The model under review builds one solid part; all positions refer to its coordinate system, in mm. A direction names the side the tool comes from. Coordinates: 2 decimals unless noted, no trailing zeros. Loops run counter-clockwise (first coordinate to the right, second up) from the corner with the lowest first, then second, coordinate; pieces in that order, holes last. Notation, with made-up numbers: M 61,60 L 76,60 A20 cw 76,97 Z; hole C 69,28.5 d7. An arc over 180 degrees is marked long. One line per item, written item: value.
```python
from build123d import *

# Parameters (mm, degrees)
BASE_PLATE_SKETCH_W        = 154
BASE_PLATE_SKETCH_H        = 154
BASE_PLATE_DEPTH           = 25
PLATE_CORNER_FILLETS_R26_R = 26
CORNER_HOLES_SKETCH_R      = 10
CORNER_HOLES_4X_20_DEPTH   = 25
CENTRAL_HUB_BOSS_DEPTH     = 31
CENTRE_TAP_DRILL_M20X2_0_D = 18
COUNTERBORE_SKETCH_R       = 14
COUNTERBORE_28_DEPTH       = 225.873297659
BORE_STEP_SKETCH_R         = 20
BORE_STEP_CUT_DEPTH        = 26
LUG_SLOT_A_SKETCH_R        = 5
LUG_SLOT_A_DEPTH           = 190.915770804
LUG_SLOT_B_SKETCH_R        = 5
LUG_SLOT_B_DEPTH           = 190.915770804
HUB_FILLETS_R12_R          = 12


with BuildPart() as part:
    # Base Plate Sketch → Base Plate (new body)
    with BuildSketch(Plane.XY):
        with Locations((77, 77)):
            Rectangle(BASE_PLATE_SKETCH_W, BASE_PLATE_SKETCH_H)
    extrude(amount=BASE_PLATE_DEPTH)

    # Plate Corner Fillets R26
    plate_corner_fillets_r26_edges = [part.edges().sort_by_distance(p)[0] for p in [
        (0, 154, 12.5),
        (154, 154, 12.5),
        (154, 0, 12.5),
        (0, 0, 12.5),
    ]]
    fillet(plate_corner_fillets_r26_edges, radius=PLATE_CORNER_FILLETS_R26_R)

    # Corner Holes Sketch → Corner Holes 4xØ20 (cut)
    with BuildSketch(Plane.XY.offset(25)):
        with Locations((26, 128)):
            Circle(CORNER_HOLES_SKETCH_R)
        with Locations((128, 128)):
            Circle(CORNER_HOLES_SKETCH_R)
        with Locations((128, 26)):
            Circle(CORNER_HOLES_SKETCH_R)
        with Locations((26, 26)):
            Circle(CORNER_HOLES_SKETCH_R)
    extrude(amount=-CORNER_HOLES_4X_20_DEPTH, mode=Mode.SUBTRACT)

    # Hub Profile Sketch → Central Hub Boss (add)
    with BuildSketch(Plane.XY.offset(25)):
        with BuildLine():
            Line((14, 58), (51.135796279, 58))
            Line((51.135796279, 58), (59.2634951, 27.931385667))
            Line((59.2634951, 27.931385667), (60.132879108, 24.715078934))
            ThreePointArc((60.132879108, 24.715078934), (77.84706214, 13.019941999), (94.383283675, 26.328656654))
            Line((94.383283675, 26.328656654), (102.894202658, 58))
            Line((102.894202658, 58), (140, 58))
            Line((140, 58), (140, 68))
            Line((140, 68), (108, 68))
            Line((108, 68), (108, 77))
            Line((108, 77), (108, 86))
            Line((108, 86), (140, 86))
            Line((140, 86), (140, 96))
            Line((140, 96), (102.894202658, 96))
            Line((102.894202658, 96), (94.383283675, 127.671343346))
            ThreePointArc((94.383283675, 127.671343346), (76.094284636, 140.977198883), (59.23523482, 125.900537557))
            Line((59.23523482, 125.900537557), (51.142468246, 96))
            Line((51.142468246, 96), (14, 96))
            Line((14, 96), (14, 86))
            Line((14, 86), (46, 86))
            Line((46, 86), (46, 77))
            Line((46, 77), (46, 68))
            Line((46, 68), (14, 68))
            Line((14, 68), (14, 58))
        make_face()
    extrude(amount=CENTRAL_HUB_BOSS_DEPTH)

    # Centre Tap Drill M20x2.0 (through all)
    with Locations(Plane.XY.offset(56)):
        with Locations((77, 123), (77, 31)):
            Hole(CENTRE_TAP_DRILL_M20X2_0_D / 2)

    # Counterbore Sketch → Counterbore Ø28 (cut, through all)
    with BuildSketch(Plane.XY.offset(56)):
        with Locations((77, 77)):
            Circle(COUNTERBORE_SKETCH_R)
    extrude(amount=-COUNTERBORE_28_DEPTH, mode=Mode.SUBTRACT)

    # Bore Step Sketch → Bore Step Cut (cut)
    with BuildSketch(Plane.XY.offset(56)):
        with Locations((77, 77)):
            Circle(BORE_STEP_SKETCH_R)
    extrude(amount=-BORE_STEP_CUT_DEPTH, mode=Mode.SUBTRACT)

    # Lug Slot A Sketch → Lug Slot A (cut, through all)
    with BuildSketch(Plane.XZ.offset(-58)):
        with Locations(Location((32.567898139, 40.5, 0), (0, 0, 270))):
            Circle(LUG_SLOT_A_SKETCH_R)
    extrude(amount=-LUG_SLOT_A_DEPTH, mode=Mode.SUBTRACT)

    # Lug Slot B Sketch → Lug Slot B (cut, through all)
    with BuildSketch(Plane.XZ.offset(-58)):
        with Locations((121.447101329, 40.5)):
            Circle(LUG_SLOT_B_SKETCH_R)
    extrude(amount=-LUG_SLOT_B_DEPTH, mode=Mode.SUBTRACT)

    # Hub Fillets R12
    hub_fillets_r12_edges = [part.edges().sort_by_distance(p)[0] for p in [
        (140, 63, 56),
        (14, 91, 56),
        (140, 91, 56),
        (14, 63, 56),
    ]]
    fillet(hub_fillets_r12_edges, radius=HUB_FILLETS_R12_R)


solid = part.part
```
(1) Draft analysis for pull direction X (two halves, no side actions). For faces 1 (the face through (55.246, 111.16, 40.283)), 2 (the face through (110, 78, 25)), 3 (the face through (72.664, 57.476, 43.182)), 4 (the face through (146.59, 146.18, 12.68)), state which applies: pulls with the +X half, pulls with the -X half, needs draft (parallel to the pull), parting line crosses it, or undercut.
Checks:
face 1: pulls with the -X half
face 2: needs draft
face 3: undercut
face 4: pulls with the +X half
(2) Insertion check: pin 1 Ø20 at (y, z) = (76, 46.5) entering from +X; pin 2 Ø5 at (y, z) = (89, 31) entering from -X; pin 3 Ø8 at (x, z) = (70.5, 38) entering from +Y. Each pin has a flat end and moves straight along its axis. Give the tip position at first contact, or say it passes through.
Checks:
pin 1: x = 140
pin 2: x = 14
pin 3: y = 140.83
(3) Add section C-C on z = 40.5. State how many separate pieces and enclosed holes the cut face has, then the cut area to 3 significant figures.
Checks:
separate pieces: 5
enclosed holes: 3
area: 4,890 mm^2
(4) Tool access review of faces 5 (the face through (76.44, 140.99, 40.28)), 6 (the face through (140, 63, 34)), 7 (the face through (14, 91, 34)): name each direction out of +Z, -Z, +X, -X, +Y, -Y from which nothing blocks a thin tool from reaching the whole face with its end or side.
Checks:
face 5: +Z, +Y
face 6: +Z, +X, +Y, -Y
face 7: +Z, -X, +Y, -Y
(5) To check wall thickness, follow L1, parallel to Y at x = 26, z = 15.5; L2, parallel to Y at x = 77, z = 14.25; L3, parallel to Y at x = 77, z = 38.25. State the ranges of each line that lie inside material, in increasing order. Write a range as [from, to].
Checks:
L1: [0, 16], [36, 118], [138, 154]
L2: [0, 22], [40, 63], [91, 114], [132, 154]
L3: [13, 22], [40, 57], [97, 114], [132, 141]
(6) Add section B-B on y = 70. State the section outline as (x, z) points (3 decimals).
Checks:
outline: M 0,0 L 64.876,0 L 64.876,30 L 58.265,30 L 58.265,56 L 46,56 L 46,25 L 0,25 Z; M 89.124,0 L 154,0 L 154,25 L 108,25 L 108,56 L 95.735,56 L 95.735,30 L 89.124,30 Z
(7) Add section D-D on x = 106. State the section outline as (y, z) points, then the cut area to 3 significant figures.
Checks:
outline: M 0,0 L 154,0 L 154,25 L 96,25 L 96,56 L 58,56 L 58,25 L 0,25 Z
area: 5,030 mm^2
(8) Add section A-A on x = 77. State the section outline as (y, z) points.
Checks:
outline: M 0,0 L 22,0 L 22,56 L 13,56 L 13,25 L 0,25 Z; M 40,0 L 63,0 L 63,30 L 57,30 L 57,56 L 40,56 Z; M 91,0 L 114,0 L 114,56 L 97,56 L 97,30 L 91,30 Z; M 132,0 L 154,0 L 154,25 L 141,25 L 141,56 L 132,56 Z
